Geometry check sheet. Reference: the model listing, model coordinates, mm. Face numbers are marked on the shaded views. A direction names the side the tool comes from. Coordinates: 2 decimals unless noted, no trailing zeros. Loops run counter-clockwise (first coordinate to the right, second up) from the corner with the lowest first, then second, coordinate; pieces in that order, holes last. Notation, with made-up numbers: (72, -31) - (98, -31) arc R14 ccw to (98, -4) - close; hole circle Ø10 at (27.5, -26). An arc over 180 degrees is marked (long way). One line per item, written item: value.
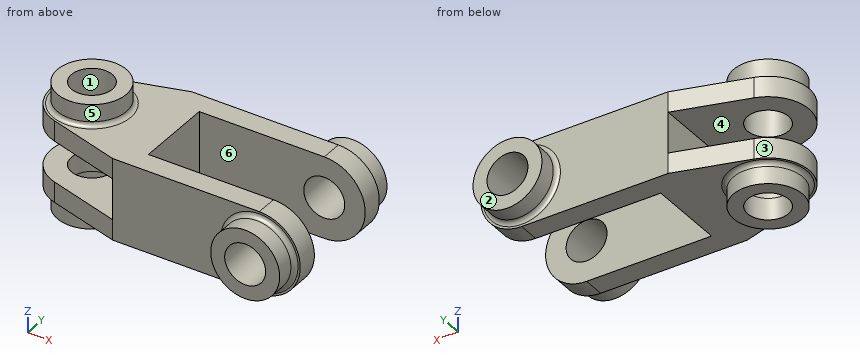
from build123d import *

# Parameters (mm, degrees)
LINK_BODY_PROFILE_SKETCH_R = 9.5
LINK_BODY_38MM_DEPTH       = 19
FORK_END_BOSS_A_SKETCH_R   = 19
FORK_END_BOSS_A_DEPTH      = 10
FORK_START                 = -10
FORK_END_BOSS_B_SKETCH_R   = 19
FORK_END_BOSS_B_DEPTH      = 10
FORK_SLOT_SKETCH_W         = 47
FORK_SLOT_SKETCH_H         = 19
FORK_SLOT_19MM_DEPTH       = 67
SIDE_HUB_SKETCH_32_R       = 16
SIDE_HUB_SKETCH_32_R_2     = 9.5
SIDE_HUB_32_DEPTH          = 10
FORK_HUB_SKETCH_32_R       = 16
FORK_HUB_32_DEPTH          = 10
FORK_PIN_BORE_SKETCH_19_R  = 9.5
FORK_PIN_BORE_19_DEPTH     = 141.861634237
EDGE_FILLETS_R2_R          = 2


with BuildPart() as part:
    # Link Body Profile Sketch → Link Body 38mm (new, symmetric)
    with BuildSketch(Plane.XY):
        with BuildLine():
            Line((-5.341003663, 18.233860806), (28, 28))
            Line((28, 28), (96, 28))
            Line((96, 28), (96, 18))
            Line((96, 18), (38, 18))
            Line((38, 18), (38, -18))
            Line((38, -18), (96, -18))
            Line((96, -18), (96, -28))
            Line((96, -28), (28, -28))
            Line((28, -28), (-5.341003663, -18.233860806))
            ThreePointArc((-5.341003663, -18.233860806), (-19, 0), (-5.341003663, 18.233860806))
        make_face()
        Circle(LINK_BODY_PROFILE_SKETCH_R, mode=Mode.SUBTRACT)
    extrude(amount=LINK_BODY_38MM_DEPTH, both=True)

    # Fork End Boss A Sketch → Fork End Boss A (add)
    with BuildSketch(Plane(origin=(0, 28, 0), x_dir=(1, 0, 0), z_dir=(0, 1, 0))):
        with Locations((96, 0)):
            Circle(FORK_END_BOSS_A_SKETCH_R)
    extrude(amount=-FORK_END_BOSS_A_DEPTH)

    # Fork End Boss B Sketch → Fork End Boss B (add)
    with BuildSketch(Plane.XZ.offset(28).offset(FORK_START)):
        with Locations((96, 0)):
            Circle(FORK_END_BOSS_B_SKETCH_R)
    extrude(amount=FORK_END_BOSS_B_DEPTH)

    # Fork Slot Sketch → Fork Slot 19mm (cut)
    with BuildSketch(Plane.XZ.offset(28)):
        with Locations((4.5, 0)):
            Rectangle(FORK_SLOT_SKETCH_W, FORK_SLOT_SKETCH_H)
    extrude(amount=-FORK_SLOT_19MM_DEPTH, mode=Mode.SUBTRACT)

    # Side Hub Sketch Ø32 → Side Hub Ø32 (add)
    with BuildSketch(Plane.XY.offset(19)):
        Circle(SIDE_HUB_SKETCH_32_R)
        Circle(SIDE_HUB_SKETCH_32_R_2, mode=Mode.SUBTRACT)
    side_hub_32 = extrude(amount=SIDE_HUB_32_DEPTH)

    # Side Hub Mirror: Side Hub Ø32 across plane
    add(side_hub_32.mirror(Plane.XY))

    # Fork Hub Sketch Ø32 → Fork Hub Ø32 (add)
    with BuildSketch(Plane(origin=(0, 28, 0), x_dir=(1, 0, 0), z_dir=(0, 1, 0))):
        with Locations((96, 0)):
            Circle(FORK_HUB_SKETCH_32_R)
    fork_hub_32 = extrude(amount=FORK_HUB_32_DEPTH)

    # Fork Hub Mirror: Fork Hub Ø32 across plane
    add(fork_hub_32.mirror(Plane.ZX))

    # Fork Pin Bore Sketch Ø19 → Fork Pin Bore Ø19 (cut, through all)
    with BuildSketch(Plane.XZ.offset(38)):
        with Locations((96, 0)):
            Circle(FORK_PIN_BORE_SKETCH_19_R)
    extrude(amount=-FORK_PIN_BORE_19_DEPTH, mode=Mode.SUBTRACT)

    # Edge Fillets R2
    edge_fillets_r2_edges = [part.edges().sort_by_distance(p)[0] for p in [
        (80, -28, 0),
        (-16, 0, 19),
        (-16, 0, -19),
        (80, 28, 0),
    ]]
    fillet(edge_fillets_r2_edges, radius=EDGE_FILLETS_R2_R)


solid = part.part
(1) Material ranges on probe 1 along Z at (x, y) = (96, -26); probe 2 along Z at (x, y) = (-9.5, 5.5); probe 3 along X at (y, z) = (0, 13.5), recorded low to high. Write a range as from..to.
Reply:
probe 1: -19..-9.5, 9.5..19
probe 2: -29..-9.5, 9.5..29
probe 3: -19..-9.5, 9.5..38
(2) Cross-section at A-A on z = 0. Record the cut outline in (x, y).
Reply:
outline: (28, -28) - (78, -28) arc R2 cw to (80, -30) - (80, -38) - (86.5, -38) - (86.5, -18) - (38, -18) - (38, 18) - (86.5, 18) - (86.5, 38) - (80, 38) - (80, 30) arc R2 cw to (78, 28) - (28, 28) - close; (105.5, -38) - (112, -38) - (112, -30) arc R2 cw to (114, -28) - (115, -28) - (115, -18) - (105.5, -18) - close; (105.5, 18) - (115, 18) - (115, 28) - (114, 28) arc R2 cw to (112, 30) - (112, 38) - (105.5, 38) - close
(3) Cross-section at C-C on x = 52. Record the cut outline in (y, z).
Reply:
outline: (-28, -19) - (-18, -19) - (-18, 19) - (-28, 19) - close; (18, -19) - (28, -19) - (28, 19) - (18, 19) - close
(4) Cross-section at B-B on y = 0. Record the cut outline in (x, z).
Reply:
outline: (-19, -19) - (-18, -19) arc R2 cw to (-16, -21) - (-16, -29) - (-9.5, -29) - (-9.5, -9.5) - (-19, -9.5) - close; (-19, 9.5) - (-9.5, 9.5) - (-9.5, 29) - (-16, 29) - (-16, 21) arc R2 cw to (-18, 19) - (-19, 19) - close; (9.5, -29) - (16, -29) - (16, -21) arc R2 cw to (18, -19) - (38, -19) - (38, 19) - (18, 19) arc R2 cw to (16, 21) - (16, 29) - (9.5, 29) - (9.5, 9.5) - (28, 9.5) - (28, -9.5) - (9.5, -9.5) - close
(5) Go/stop test with flat-tipped pins: pin 1 Ø4 at (x, z) = (45.5, 3.5) entering from -Y; pin 2 Ø2 at (y, z) = (26.5, -21) entering from -X; pin 3 Ø19 at (x, z) = (59, 7) entering from +Y; pin 4 Ø17 at (x, y) = (24.5, 6) entering from +Z. Record where each tip stops, or that it passes through.
Reply:
pin 1: y = -28
pin 2: through
pin 3: y = 28
pin 4: z = 19.46
(6) Cross-section at D-D on x = 0. Record the cut outline in (y, z), and give its area (3 significant figures).
Reply:
outline: (-19.8, -19) - (-18, -19) arc R2 cw to (-16, -21) - (-16, -29) - (-9.5, -29) - (-9.5, -9.5) - (-19.8, -9.5) - close; (-19.8, 9.5) - (-9.5, 9.5) - (-9.5, 29) - (-16, 29) - (-16, 21) arc R2 cw to (-18, 19) - (-19.8, 19) - close; (9.5, -29) - (16, -29) - (16, -21) arc R2 cw to (18, -19) - (19.8, -19) - (19.8, -9.5) - (9.5, -9.5) - close; (9.5, 9.5) - (19.8, 9.5) - (19.8, 19) - (18, 19) arc R2 cw to (16, 21) - (16, 29) - (9.5, 29) - close
area: 655 mm2
(7) Access from +Z, -Z, +X, -X, +Y, -Y to the whole of each face (thin tool, end or side, straight path). Record for the marked faces 4, 5 and 6.
Reply:
face 4: -X, +Y, -Y
face 5: +Z
face 6: +Z, -Z, +X
(8) Release check for a two-part mould opening along X. For the marked faces 1, 2 and 3 record: pulls with the +X half, pulls with the -X half, needs draft (parallel to the pull), parting line crosses it, or undercut.
Reply:
face 1: undercut
face 2: needs draft
face 3: pulls with the -X half
